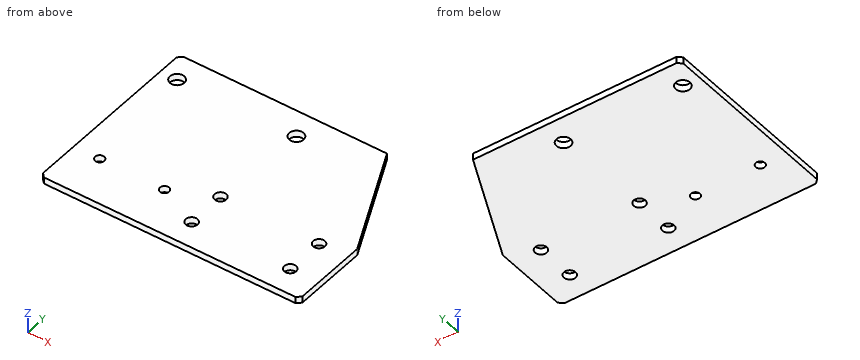
```python
from build123d import *

# Parameters (mm, degrees)
SKETCH_1_R      = 4.5
SKETCH_1_R_2    = 3.5
SKETCH_1_R_3    = 5.5
EXTRUDE_1_DEPTH = 5


with BuildPart() as part:
    # 草图1 → 凸台-拉伸1 (new body)
    with BuildSketch(Plane.XY.offset(2.5)):
        Polygon((-97, -72.5), (97, -72.5), (100, -69.5), (100, -12.5), (60, 72.5), (-97, 72.5), (-100, 69.5), (-100, -69.5), align=None)
        with Locations(Location((2, -22.5, 0), (0, 0, 180))):
            Circle(SKETCH_1_R, mode=Mode.SUBTRACT)
        with Locations(Location((-30, -37.5, 0), (0, 0, 180))):
            Circle(SKETCH_1_R_2, mode=Mode.SUBTRACT)
        with Locations(Location((-80, -37.5, 0), (0, 0, 180))):
            Circle(SKETCH_1_R_2, mode=Mode.SUBTRACT)
        with Locations(Location((5, 52.5, 0), (0, 0, 180))):
            Circle(SKETCH_1_R_3, mode=Mode.SUBTRACT)
        with Locations(Location((78, -52.5, 0), (0, 0, 180))):
            Circle(SKETCH_1_R, mode=Mode.SUBTRACT)
        with Locations(Location((2, -52.5, 0), (0, 0, 180))):
            Circle(SKETCH_1_R, mode=Mode.SUBTRACT)
        with Locations(Location((78, -22.5, 0), (0, 0, 180))):
            Circle(SKETCH_1_R, mode=Mode.SUBTRACT)
        with Locations(Location((-87, 52.5, 0), (0, 0, 180))):
            Circle(SKETCH_1_R_3, mode=Mode.SUBTRACT)
    extrude(amount=-EXTRUDE_1_DEPTH)


solid = part.part
```
CAD build for the part. Positions are in the model's coordinates, mm. Give positions to 0.01 mm unless a question says otherwise; leave off trailing zeros. Order: outer loops, then holes, each group sorted by start corner. A loop starts at its lowest first (then second) coordinate and runs counter-clockwise, first axis right, second up.
(1) Saw through at B-B, the plane y = -52.5. Give the cut face in (x, z), then the cut area to 3 significant figures.
(2) Flat gauge pin, fed straight in: pin 1 (5.5 mm diameter, centred on x = -80, y = -37.5, fed in from +Z). Where does the tip first touch, or does it go through?
(3) Saw through at C-C, the plane x = 2. Give the cut face in (y, z), then the cut area to 3 significant figures.
(4) Saw through at A-A, the plane x = -30. Give the cut face in (y, z), then the cut area to 3 significant figures.
(5) Saw through at D-D, the plane z = 0.4. State how many separate pieces and enclosed holes the cut face has, then the cut area to 3 significant figures.
(6) Drill centre lines: L1, parallel to X at y = -23, z = 0.75; L2, parallel to Y at x = -80, z = 1.05; L3, parallel to Y at x = 5, z = 1.05. Where is each one in solid material? Low to high.
Results found:
1. outline: (-100, -2.5) - (-2.5, -2.5) - (-2.5, 2.5) - (-100, 2.5) - close; (6.5, -2.5) - (73.5, -2.5) - (73.5, 2.5) - (6.5, 2.5) - close; (82.5, -2.5) - (100, -2.5) - (100, 2.5) - (82.5, 2.5) - close
1. area: 910 mm2
2. pin 1: passes through
3. outline: (-72.5, -2.5) - (-57, -2.5) - (-57, 2.5) - (-72.5, 2.5) - close; (-48, -2.5) - (-27, -2.5) - (-27, 2.5) - (-48, 2.5) - close; (-18, -2.5) - (47.89, -2.5) - (47.89, 2.5) - (-18, 2.5) - close; (57.11, -2.5) - (72.5, -2.5) - (72.5, 2.5) - (57.11, 2.5) - close
3. area: 589 mm2
4. outline: (-72.5, -2.5) - (-41, -2.5) - (-41, 2.5) - (-72.5, 2.5) - close; (-34, -2.5) - (72.5, -2.5) - (72.5, 2.5) - (-34, 2.5) - close
4. area: 690 mm2
5. separate pieces: 1
5. enclosed holes: 8
5. area: 26,800 mm2
6. L1: x = -100 to -2.47, 6.47 to 73.53, 82.47 to 100
6. L2: y = -72.5 to -41, -34 to 72.5
6. L3: y = -72.5 to -55.85, -49.15 to -25.85, -19.15 to 47, 58 to 72.5
